The model under review builds one solid part; all positions refer to its coordinate system, in mm. Round coordinates to 2 decimals unless told otherwise and drop trailing zeros. Loops run counter-clockwise (first coordinate to the right, second up) from the corner with the lowest first, then second, coordinate; pieces in that order, holes last. Notation, with made-up numbers: M -5,25.5 L 0,25.5 A27 cw 0,42.5 Z; hole C 46.5,43 d2. An arc over 180 degrees is marked long. Answer as a JSON object with one key per item and string values. Group by question number.
Item 1: Insertion check: P1, Ø5, axis at x = 61.13, y = -84.14, coming from the +Z side; P2, Ø4, axis at x = 0, y = 104, coming from the +Z side; P3, Ø1.5, axis at y = 60, z = 1, coming from the -X side; P4, Ø2, axis at y = 1.5, z = 1, coming from the +X side. Each pin has a flat end and moves straight along its axis. Give the tip position at first contact, or say it passes through.
Item 2: Consider section B-B (x = 44.5). Give the boundary of the cut face in (y, z).
Item 3: The part is to be moulded in two halves that separate along Y. For faces 1 (the face through (-23.846, -107.384, 1.972)), 2 (the face through (100.357, 34.025, 2.078)), 3 (the face through (23, -47, 4)), say which applies: +Y half, -Y half, draft (parallel to the pull), parting line (faces both ways), or undercut.
Item 4: To check wall thickness, follow line 1 (Y direction, x = 0, z = 1); line 2 (X direction, y = 33, z = 1.15); line 3 (X direction, y = 1, z = 0.9). State the ranges of each line that lie inside material, in increasing order.
Item 5: Consider section D-D (y = 89). Give the boundary of the cut face in (x, z).
Item 6: Consider section A-A (y = 0). Give the boundary of the cut face in (x, z), and give its area (3 significant figures).
Item 7: Consider section C-C (z = 1.1). Give the boundary of the cut face in (x, y).
```python
from build123d import *

# Parameters (mm, degrees)
SKETCH1_R                                 = 110
SKETCH1_R_2                               = 50
BOSS_EXTRUDE1_DEPTH                       = 4
HOLE_SIZE_PER_CROSS_SLOTTED_COUNT_2_COUNT = 2
HOLE_SIZE_PER_CROSS_SLOTTED_COUNT_2_PITCH = 122.259332477
HOLE_SIZE_PER_CROSS_SLOTTED_COUNT_3_COUNT = 2
HOLE_SIZE_PER_CROSS_SLOTTED_COUNT_3_PITCH = 197.819755389
HOLE_SIZE_PER_CROSS_SLOTTED_COUNT_4_COUNT = 2
HOLE_SIZE_PER_CROSS_SLOTTED_COUNT_4_PITCH = 197.819755389
HOLE_SIZE_PER_CROSS_SLOTTED_COUNT_5_COUNT = 2
HOLE_SIZE_PER_CROSS_SLOTTED_COUNT_5_PITCH = 122.259332477


with BuildPart() as part:
    # Sketch1 → Boss-Extrude1 (new body)
    with BuildSketch(Plane.XY):
        Circle(SKETCH1_R)
        Circle(SKETCH1_R_2, mode=Mode.SUBTRACT)
    extrude(amount=BOSS_EXTRUDE1_DEPTH)

    # Sketch5 → Hole Size (% per cross) Slotted Countersunk Wood Screw Type1 (revolve, cut)
    with BuildSketch(Plane(origin=(0, 104, 4), x_dir=(0, -1, 0), z_dir=(1, 0, 0))):
        Polygon((0, 0), (0, 4), (2.25, 4), (2.25, 2.05), (4.3, 0), align=None)
    hole_size_per_cross_slotted_countersu = revolve(axis=Axis((0, 104, 10.35), (0, 0, -1)), mode=Mode.SUBTRACT)

    # Hole Size _ per cross_ Slotted Count 2: Hole Size (% per cross) Slotted Countersunk Wood Screw Type1 ×2
    with Locations(*[Vector(0.8090169943749717, -0.5877852522924399, 0) * (i * HOLE_SIZE_PER_CROSS_SLOTTED_COUNT_2_PITCH) for i in range(1, HOLE_SIZE_PER_CROSS_SLOTTED_COUNT_2_COUNT)]):
        add(hole_size_per_cross_slotted_countersu, mode=Mode.SUBTRACT)

    # Hole Size _ per cross_ Slotted Count 3: Hole Size (% per cross) Slotted Countersunk Wood Screw Type1 ×2
    with Locations(*[Vector(0.3090169943749865, -0.9510565162951409, 0) * (i * HOLE_SIZE_PER_CROSS_SLOTTED_COUNT_3_PITCH) for i in range(1, HOLE_SIZE_PER_CROSS_SLOTTED_COUNT_3_COUNT)]):
        add(hole_size_per_cross_slotted_countersu, mode=Mode.SUBTRACT)

    # Hole Size _ per cross_ Slotted Count 4: Hole Size (% per cross) Slotted Countersunk Wood Screw Type1 ×2
    with Locations(*[Vector(-0.30901699437490837, -0.9510565162951663, 0) * (i * HOLE_SIZE_PER_CROSS_SLOTTED_COUNT_4_PITCH) for i in range(1, HOLE_SIZE_PER_CROSS_SLOTTED_COUNT_4_COUNT)]):
        add(hole_size_per_cross_slotted_countersu, mode=Mode.SUBTRACT)

    # Hole Size _ per cross_ Slotted Count 5: Hole Size (% per cross) Slotted Countersunk Wood Screw Type1 ×2
    with Locations(*[Vector(-0.8090169943749234, -0.5877852522925062, 0) * (i * HOLE_SIZE_PER_CROSS_SLOTTED_COUNT_5_PITCH) for i in range(1, HOLE_SIZE_PER_CROSS_SLOTTED_COUNT_5_COUNT)]):
        add(hole_size_per_cross_slotted_countersu, mode=Mode.SUBTRACT)


solid = part.part
```
Geometry results:
{
 "1": {"P1": "stops at z = 2.2", "P2": "passes through", "P3": "stops at x = -92.68", "P4": "stops at x = 110"},
 "2": {"outline": "M -100.6,0 L -22.8,0 L -22.8,4 L -100.6,4 Z; M 22.8,0 L 100.6,0 L 100.6,4 L 22.8,4 Z"},
 "3": {"face 1": "parting line", "face 2": "undercut", "face 3": "draft"},
 "4": {"line 1": "y = -110 to -50, 50 to 101.75, 106.25 to 110", "line 2": "x = -104.93 to -100.99, -96.83 to -37.56, 37.56 to 96.83, 100.99 to 104.93", "line 3": "x = -110 to -49.99, 49.99 to 110"},
 "5": {"outline": "M -64.65,0 L 64.65,0 L 64.65,4 L -64.65,4 Z"},
 "6": {"outline": "M -110,0 L -50,0 L -50,4 L -110,4 Z; M 50,0 L 110,0 L 110,4 L 50,4 Z", "area": "480 mm^2"},
 "7": {"outline": "C 0,0 d220; hole C -98.91,32.14 d4.5; hole C -61.13,-84.14 d4.5; hole C 0,0 d100; hole C 0,104 d4.5; hole C 61.13,-84.14 d4.5; hole C 98.91,32.14 d4.5"}
}
